Geometry: final body of the model. Coordinates: model frame, mm. Coordinates: 2 decimals unless noted, no trailing zeros. Write each loop counter-clockwise with the first axis right and the second up, starting at its lowest first coordinate (ties: lowest second). Pieces come first, ordered by that corner, then holes. Notation, with made-up numbers: (-33, -28.75) - (-10, -28.75) arc R18 ccw to (-10, -10.75) - close; hole circle Ø8 at (8.5, -36). An arc over 180 degrees is marked (long way). Put each result on its own line as item: value.
```python
from build123d import *

# Parameters (mm, degrees)
BOSS_EXTRUDE1_DEPTH     = 12.5
CUT_EXTRUDE1_DEPTH      = 768.828594154
CUT_EXTRUDE1_DEPTH_BACK = 768.828594154
SKETCH2_R               = 60.5
SKETCH2_R_2             = 66.5
FILLET1_R               = 70
CHAMFER1_SIZE           = 12
CHAMFER2_SIZE           = 12
CUT_EXTRUDE2_DEPTH      = 65
CUT_EXTRUDE3_DEPTH      = 95


with BuildPart() as part:
    # Sketch1 → Boss-Extrude1 (new, symmetric)
    with BuildSketch(Plane(origin=(0, 0, 0), x_dir=(0, 0, -1), z_dir=(1, 0, 0))):
        with BuildLine():
            Line((-161.139129372, 353.5), (152.4, 353.5))
            ThreePointArc((152.4, 353.5), (215.520549571, 325.671884154), (237.552772458, 260.302250804))
            ThreePointArc((237.552772458, 260.302250804), (255.590849676, 206.783252739), (307.268492599, 184))
            Line((307.268492599, 184), (515.051943832, 184))
            ThreePointArc((515.051943832, 184), (651.90709321, 177.635326105), (657.753510977, 40.757057617))
            Line((657.753510977, 40.757057617), (624.56119852, 1.2))
            Line((624.56119852, 1.2), (252.997154134, 1.2))
            ThreePointArc((252.997154134, 1.2), (0, 253), (-252.997154134, 1.2))
            Line((-252.997154134, 1.2), (-624, 1.2))
            Line((-624, 1.2), (-667.696816027, 138.145895408))
            ThreePointArc((-667.696816027, 138.145895408), (-594.001115997, 267.859489493), (-470.614493078, 184))
            Line((-470.614493078, 184), (-259, 184))
            Line((-259, 184), (-161.139129372, 353.5))
        make_face()
    extrude(amount=BOSS_EXTRUDE1_DEPTH, both=True)

    # Sketch2 → Cut-Extrude1 (cut, two sides: drawn at the far end of the back side and taken through both)
    with BuildSketch(Plane(origin=(0, 0, 0), x_dir=(0, 0, -1), z_dir=(1, 0, 0)).offset(-CUT_EXTRUDE1_DEPTH_BACK)):
        with Locations((152.4, 268)):
            Circle(SKETCH2_R)
        with Locations((-571, 169)):
            Circle(SKETCH2_R_2)
        with Locations((580, 106)):
            Circle(SKETCH2_R_2)
    extrude(amount=CUT_EXTRUDE1_DEPTH + CUT_EXTRUDE1_DEPTH_BACK, mode=Mode.SUBTRACT)

    # Fillet1
    fillet1_edges = [part.edges().sort_by_distance(p)[0] for p in [
        (0, 184, 470.614493078),
        (0, 184, 259),
        (0, 353.5, 161.139129372),
        (0, 184, -515.051943832),
    ]]
    fillet(fillet1_edges, radius=FILLET1_R)

    # Chamfer1
    chamfer1_edges = [part.edges().sort_by_distance(p)[0] for p in [
        (12.5, 213.213707904, 136.194400626),
        (12.5, 118.018425376, -223.787066811),
        (12.5, 320.591390839, -182.306447626),
        (12.5, 169, 637.5),
        (12.5, 106, -513.5),
    ]]
    chamfer(chamfer1_edges, length=CHAMFER1_SIZE)

    # Chamfer2
    chamfer2_edges = [part.edges().sort_by_distance(p)[0] for p in [
        (-12.5, 1.2, -438.779176327),
        (-12.5, 1.2, 438.498577067),
    ]]
    chamfer(chamfer2_edges, length=CHAMFER2_SIZE)

    # Sketch3 → Cut-Extrude2 (cut, symmetric)
    with BuildSketch(Plane.XY.offset(360)):
        Polygon((5.5, 190), (-12.5, 172), (-12.5, 190), align=None)
    extrude(amount=CUT_EXTRUDE2_DEPTH, both=True, mode=Mode.SUBTRACT)

    # Sketch4 → Cut-Extrude3 (cut, symmetric)
    with BuildSketch(Plane.XY.offset(-400)):
        Polygon((-12.5, 172), (5.5, 190), (-12.5, 190), align=None)
    extrude(amount=CUT_EXTRUDE3_DEPTH, both=True, mode=Mode.SUBTRACT)


solid = part.part
```
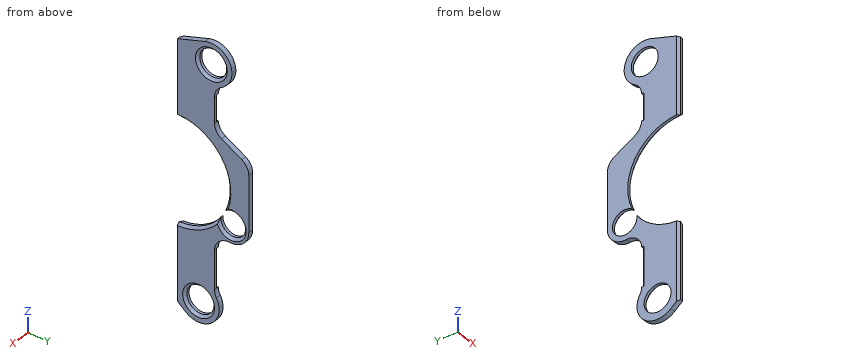
1. Section query D-D (z = 391). Return loops of the section in (x, y).
Answer below:
outline: (-12.5, 13.2) - (-0.5, 1.2) - (12.5, 1.2) - (12.5, 184) - (-0.5, 184) - (-12.5, 172) - close
2. Pin query (flat end, axial travel): pin 1 Ø2 at (x, y) = (-5, 136) entering from +Z; pin 2 Ø6 at (x, y) = (-7.5, 179) entering from -Z; pin 3 Ø10 at (x, z) = (4, -280.5) entering from +Y. Return the tip coordinate at first contact, or that it passes through.
Answer below:
pin 1: stops at z = 667.33
pin 2: stops at z = -653.5
pin 3: stops at y = 191.62
3. Ray query, probe 1 along Z at (x, y) = (-11, 62); probe 2 along Z at (x, y) = (11.25, 134.5); probe 3 along Z at (x, y) = (6.75, 223). Return the intervals inside material, ascending. Write a range as from..to.
Answer below:
probe 1: z = -671.47..-629.86, -530.14..-245.29, 245.29..643.4
probe 2: z = -677.42..-651.8, -508.2..-226.88, 226.88..501.88, 640.12..666.53
probe 3: z = -244.51..-201.7, 132.22..236.48, 485.06..522.25, 619.75..656.94
4. Section query A-A (z = -580). Return loops of the section in (x, y), then the cut area to 3 significant figures.
Answer below:
outline: (-12.5, 13.2) - (-0.5, 1.2) - (12.5, 1.2) - (12.5, 27.5) - (0.5, 39.5) - (-12.5, 39.5) - close; (-12.5, 172.5) - (0.5, 172.5) - (12.5, 184.5) - (12.5, 207.5) - (-12.5, 207.5) - close
area: 1,620 mm²
5. Section query B-B (x = -7.5). Return loops of the section in (y, z), then the cut area to 3 significant figures.
Answer below:
outline: (8.2, -630.43) - (40.76, -657.75) arc R101.5 ccw to (193.59, -528.72) arc R70 cw to (184.02, -495) - (177, -495) - (177, -305) - (184.04, -305) arc R70 cw to (260.3, -237.55) arc R85.5 ccw to (353.5, -152.4) - (353.5, 120.72) arc R70 ccw to (318.5, 181.35) - (219, 238.79) arc R70 cw to (184.14, 295) - (177, 295) - (177, 425) - (184.06, 425) arc R70 cw to (219.31, 482.84) arc R101.5 ccw to (138.15, 667.7) - (8.2, 626.23) - (8.2, 252.87) arc R253 cw to (230.06, -105.28) arc R60.5 cw (long way) to (208.1, -143.88) arc R253 cw to (8.2, -252.87) - close; hole circle Ø133 at (106, -580); hole circle Ø133 at (169, 571)
area: 185,000 mm²
6. Section query C-C (z = 571). Return loops of the section in (x, y).
Answer below:
outline: (-12.5, 13.2) - (-0.5, 1.2) - (12.5, 1.2) - (12.5, 90.5) - (0.5, 102.5) - (-12.5, 102.5) - close; (-12.5, 235.5) - (0.5, 235.5) - (12.5, 247.5) - (12.5, 270.5) - (-12.5, 270.5) - close
